The model under review builds one solid part; all positions refer to its coordinate system, in mm. Give positions to 0.01 mm unless a question says otherwise; leave off trailing zeros. Loops run counter-clockwise (first coordinate to the right, second up) from the corner with the lowest first, then second, coordinate; pieces in that order, holes last. Notation, with made-up numbers: M 73,-25 L 88,-25 A21 cw 88,12 Z; hole C 74.5,13.5 d2. An arc over 180 degrees is marked long. Return JSON: item names as keys, results as strings.
```python
from build123d import *

# Parameters (mm, degrees)
BOSS_EXTRUDE1_DEPTH = 8
CHAMFER1_SIZE       = 5


with BuildPart() as part:
    # Sketch1 → Boss-Extrude1 (new body)
    with BuildSketch(Plane.XY):
        Polygon((0, 80), (0, 0), (80, 0), (80, 10), (10, 80), align=None)
    extrude(amount=BOSS_EXTRUDE1_DEPTH)

    # Chamfer1
    chamfer1_edges = [part.edges().sort_by_distance(p)[0] for p in [
        (0, 0, 4),
    ]]
    chamfer(chamfer1_edges, length=CHAMFER1_SIZE)


solid = part.part
```
1) Consider section A-A on y = 36. Write out the cut boundary in (x, z), then the cut area to 3 significant figures.
From the geometry:
{"outline": "M 0,0 L 54,0 L 54,8 L 0,8 Z", "area": "432 mm²"}
2) Wall thickness on L1, parallel to X at y = 21.5, z = 2; L2, parallel to X at y = 66, z = 4.25; L3, parallel to Y at x = 4, z = 1.25: over which ranges is each line inside the solid? List them lowest first. Write a range as from..to.
From the geometry:
{"L1": "0..68.5", "L2": "0..24", "L3": "1..80"}
3) Consider section B-B on z = 4.75. Write out the cut boundary in (x, y).
From the geometry:
{"outline": "M 0,5 L 5,0 L 80,0 L 80,10 L 10,80 L 0,80 Z"}
4) Consider section C-C on x = 61. Write out the cut boundary in (y, z), then the cut area to 3 significant figures.
From the geometry:
{"outline": "M 0,0 L 29,0 L 29,8 L 0,8 Z", "area": "232 mm²"}
